Check sheet for the modelled part. Datum: model origin and axes. Units: mm. Coordinates: 2 decimals unless noted, no trailing zeros. Order: outer loops, then holes, each group sorted by start corner. A loop starts at its lowest first (then second) coordinate and runs counter-clockwise, first axis right, second up.
from build123d import *

# Parameters (mm, degrees)
SKETCH1_W                  = 200
SKETCH1_H                  = 80
BOSS_EXTRUDE1_DEPTH        = 10
F_6_6_6_6_DIAMETER_HOLE1_D = 6.6


with BuildPart() as part:
    # Sketch1 → Boss-Extrude1 (new body)
    with BuildSketch(Plane(origin=(0, 0, 0), x_dir=(1, 0, 0), z_dir=(0, 1, 0))):
        Rectangle(SKETCH1_W, SKETCH1_H)
    extrude(amount=BOSS_EXTRUDE1_DEPTH)

    # Ø6.6 (6.6) Diameter Hole1 (through all)
    with Locations(Plane(origin=(0, 10, 0), x_dir=(1, 0, 0), z_dir=(0, 1, 0))):
        with Locations((-25, 25), (25, 25), (-25, -25), (25, -25), (-75, 25), (75, 25), (75, -25), (-75, -25)):
            Hole(F_6_6_6_6_DIAMETER_HOLE1_D / 2)


solid = part.part
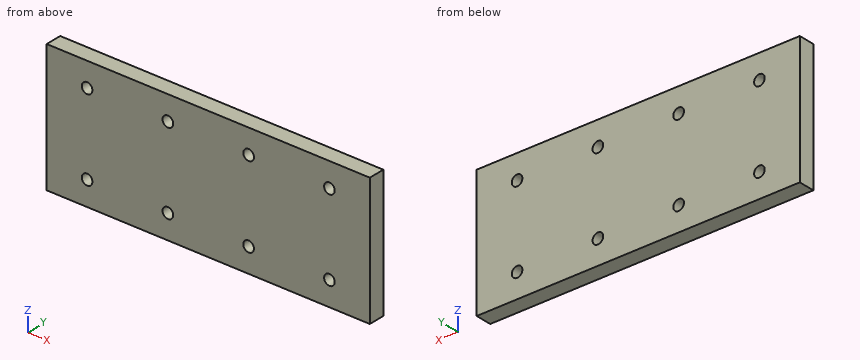
(1) Cross-section at C-C (z = 25). Enter the section's corners in (x, y).
Filled in:
outline: (-100, 0) - (-78.3, 0) - (-78.3, 10) - (-100, 10) - close; (-71.7, 0) - (-28.3, 0) - (-28.3, 10) - (-71.7, 10) - close; (-21.7, 0) - (21.7, 0) - (21.7, 10) - (-21.7, 10) - close; (28.3, 0) - (71.7, 0) - (71.7, 10) - (28.3, 10) - close; (78.3, 0) - (100, 0) - (100, 10) - (78.3, 10) - close
(2) Cross-section at A-A (x = 25). Enter the section's corners in (y, z).
Filled in:
outline: (0, -40) - (10, -40) - (10, -28.3) - (0, -28.3) - close; (0, -21.7) - (10, -21.7) - (10, 21.7) - (0, 21.7) - close; (0, 28.3) - (10, 28.3) - (10, 40) - (0, 40) - close
(3) Thickness scan on probe 1 along X at (y, z) = (7.25, 25); probe 2 along Z at (x, y) = (-25, 3.25); probe 3 along X at (y, z) = (2.75, -26). Record the ranges inside material, lowest first.
Filled in:
probe 1: x = -100 to -78.3, -71.7 to -28.3, -21.7 to 21.7, 28.3 to 71.7, 78.3 to 100
probe 2: z = -40 to -28.3, -21.7 to 21.7, 28.3 to 40
probe 3: x = -100 to -78.14, -71.86 to -28.14, -21.86 to 21.86, 28.14 to 71.86, 78.14 to 100
(4) Go/stop test with flat-tipped pins: P1, Ø5.5, axis at x = -25, z = 25, coming from the +Y side; P2, Ø8.5, axis at x = -75, z = 25, coming from the -Y side. Record where each tip stops, or that it passes through.
Filled in:
P1: passes through
P2: stops at y = 0
(5) Cross-section at B-B (y = 6.5). Count the separate pieces of the cut face and the enclosed holes in it, and give its area (3 significant figures).
Filled in:
separate pieces: 1
enclosed holes: 8
area: 15,700 mm2
